from build123d import *

# Parameters (mm, degrees)
SKETCH1_R             = 6
BOSS_EXTRUDE1_DEPTH   = 160
M6_TAPPED_HOLE1_D     = 5
M6_TAPPED_HOLE1_DEPTH = 15
M6_TAPPED_HOLE1_TIP   = 1.502151548
CHAMFER1_SIZE         = 0.5


with BuildPart() as part:
    # Sketch1 → Boss-Extrude1 (new body)
    with BuildSketch(Plane.XY):
        Circle(SKETCH1_R)
    extrude(amount=BOSS_EXTRUDE1_DEPTH)

    # M6 Tapped Hole1
    with Locations(Plane.XY.offset(160)):
        with Locations((0, 0)):
            Hole(M6_TAPPED_HOLE1_D / 2, depth=M6_TAPPED_HOLE1_DEPTH)
            with Locations((0, 0, -(M6_TAPPED_HOLE1_DEPTH + M6_TAPPED_HOLE1_TIP / 2))):  # 118° drill point
                Cone(0, M6_TAPPED_HOLE1_D / 2, M6_TAPPED_HOLE1_TIP, mode=Mode.SUBTRACT)

    # Chamfer1
    chamfer1_edges = [part.edges().sort_by_distance(p)[0] for p in [
        (-6, 0, 0),
        (-6, 0, 160),
    ]]
    chamfer(chamfer1_edges, length=CHAMFER1_SIZE)


solid = part.part
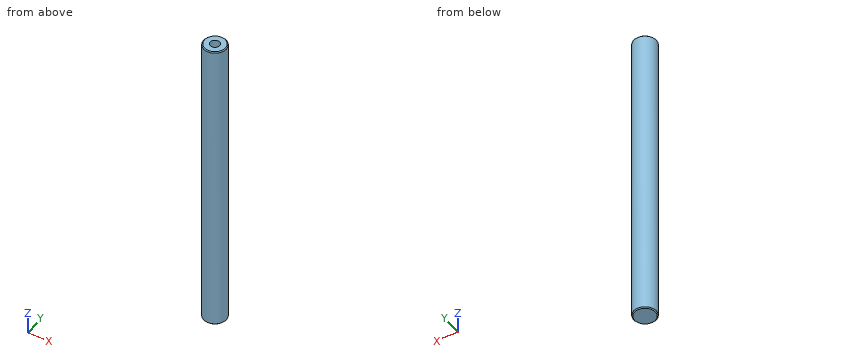
Build history of the part. All positions in model axes, mm. Round coordinates to 2 decimals unless told otherwise and drop trailing zeros. Write each loop counter-clockwise with the first axis right and the second up, starting at its lowest first coordinate (ties: lowest second). Pieces come first, ordered by that corner, then holes. Notation, with made-up numbers: (68.5, -17) - (112.5, -17) arc R18 cw to (112.5, 0) - close; hole circle Ø10 at (18.5, 22). An arc over 180 degrees is marked (long way). Use CSV: the item, a comma, the result in double quotes.
(1) Band-saw the part on A-A (z = 127.5). Write the cut outline in (x, y).
Response:
outline,"circle Ø12 at (0, 0)"
(2) Band-saw the part on B-B (z = 148.5). Write the cut outline in (x, y), plus the area to 3 significant figures.
Response:
outline,"circle Ø12 at (0, 0); hole circle Ø5 at (0, 0)"
area,"93.5 mm²"
(3) Wall check: line 1 (Y direction, x = 0, z = 155.5); line 2 (X direction, y = -3.5, z = 50); line 3 (Z direction, x = -1.25, y = 0.75). Give the ranges that are in metal, low to high.
Response:
line 1,"-6 to -2.5, 2.5 to 6"
line 2,"-4.87 to 4.87"
line 3,"0 to 144.37"
(4) Pin check, flat tips, straight feed: P1, Ø4, axis at y = -2.5, z = 76, coming from the -X side; P2, Ø5, axis at x = -3.5, z = 103, coming from the +Y side; P3, Ø1, axis at x = -3.5, z = 90, coming from the +Y side. Stop position of each tip, or through.
Response:
P1,"x = -5.98"
P2,"y = 5.92"
P3,"y = 5.2"
